Here's how the part is built. I have some questions about the finished solid (model axes, mm). A direction names the side the tool comes from. Coordinates: 2 decimals unless noted, no trailing zeros. Loops run counter-clockwise (first coordinate to the right, second up) from the corner with the lowest first, then second, coordinate; pieces in that order, holes last. Notation, with made-up numbers: (63, 80) -> (107, 80) arc R17 ccw to (107, 108) -> close; hole circle Ø11 at (48.25, 45.5). An arc over 180 degrees is marked (long way). Answer as a JSON object with one key per item and string values. Group by question number.
Q1. On a 3-axis mill with a long thin cutter (end or side, diameter ignored), from which of +Z, -Z, +X, -X, +Y, -Y can I reach the whole of each face in a straight line? I mean faces 4 (the flat face through (24, 0, -5)), 5 (the flat face through (97.93, 6.14, 0.04)), 6 (the flat face through (97.812, -6.107, 0.042)). Say none if no direction works.
Q2. I need wall thicknesses on line 1 (Y direction, x = 104, z = -0.7); line 2 (Y direction, x = 0, z = 3); line 3 (X direction, y = -1, z = 4.25). Which ranges of each line are inside material? Lowest first, please.
Q3. I want a section at D-D on x = 58. Write out the boundary of the cut face in (y, z).
Q4. I'm going to push flat-ended pins straight in: pin 1 (1 mm diameter, centred on y = -15, z = -1.5, fed in from +X); pin 2 (1.6 mm diameter, centred on y = 1.5, z = 3.5, fed in from +X); pin 3 (4.5 mm diameter, centred on x = 96.5, y = 0, fed in from -Z); pin 4 (5.5 mm diameter, centred on x = 104, y = 0, fed in from -Z). Where does each tip first touch, or does it pass through?
Q5. Thinking about a two-plate mould opening in X: for faces 1 (the flat face through (-19.7, 19.9, 0.1)), 2 (the flat face through (64, -5, 0)), 3 (the flat face through (0, 28, 0)), which applies, released by +X, released by -X, zero draft, split by the parting line, or undercut?
Q6. I want a section at A-A on x = 0. Write out the boundary of the cut face in (y, z).
Q7. I want a section at C-C on y = 9.5. Write out the boundary of the cut face in (x, z), then the cut area to 3 significant figures.
Q8. I want a section at B-B on z = -1.25. Write out the boundary of the cut face in (x, y), then the cut area to 3 significant figures.
```python
from build123d import *

# Parameters (mm, degrees)
SKETCH_1_3_R        = 22.5
BOSS_EXTRUDE1_DEPTH = 5
BOSS_EXTRUDE2_DEPTH = 3
SKETCH2_R           = 3
CUT_EXTRUDE1_DEPTH  = 15.5


with BuildPart() as part:
    # Sketch 1_3 → Boss-Extrude1 (new, symmetric)
    with BuildSketch(Plane.XY):
        Polygon((34.597979746, 5), (28, 11.597979746), (11.597979746, 28), (-11.597979746, 28), (-28, 11.597979746), (-28, -11.597979746), (-11.597979746, -28), (11.597979746, -28), (19.798989873, -19.798989873), (28, -11.597979746), (34.597979746, -5), (82, -5), (84, -3), (84, 3), (82, 5), align=None)
        Circle(SKETCH_1_3_R, mode=Mode.SUBTRACT)
    extrude(amount=BOSS_EXTRUDE1_DEPTH, both=True)

    # Sketch 1_3 2 → Boss-Extrude2 (add, symmetric)
    with BuildSketch(Plane.XY):
        with BuildLine():
            Line((93.682479249, 5), (82, 5))
            Line((82, 5), (84, 3))
            Line((84, 3), (84, -3))
            Line((84, -3), (82, -5))
            Line((82, -5), (93.682479249, -5))
            Line((93.682479249, -5), (102.058857162, -7.244443697))
            ThreePointArc((102.058857162, -7.244443697), (111.5, 0), (102.058857162, 7.244443697))
            Line((102.058857162, 7.244443697), (93.682479249, 5))
        make_face()
    extrude(amount=BOSS_EXTRUDE2_DEPTH, both=True)

    # Sketch2 → Cut-Extrude1 (cut, symmetric)
    with BuildSketch(Plane.XY.offset(3)):
        with Locations((104, 0)):
            Circle(SKETCH2_R)
    extrude(amount=CUT_EXTRUDE1_DEPTH, both=True, mode=Mode.SUBTRACT)


solid = part.part
```
Result set:
{
 "1": {"face 4": "-Z, +X, -X, +Y, -Y", "face 5": "+Z, -Z, +Y", "face 6": "+Z, -Z, -Y"},
 "2": {"line 1": "y = -7.5 to -3, 3 to 7.5", "line 2": "y = -28 to -22.5, 22.5 to 28", "line 3": "x = -28 to -22.48, 22.48 to 84"},
 "3": {"outline": "(-5, -5) -> (5, -5) -> (5, 5) -> (-5, 5) -> close"},
 "4": {"pin 1": "stops at x = 25.1", "pin 2": "stops at x = 111.45", "pin 3": "stops at z = -3", "pin 4": "passes through"},
 "5": {"face 1": "released by -X", "face 2": "undercut", "face 3": "zero draft"},
 "6": {"outline": "(-28, -5) -> (-22.5, -5) -> (-22.5, 5) -> (-28, 5) -> close; (22.5, -5) -> (28, -5) -> (28, 5) -> (22.5, 5) -> close"},
 "7": {"outline": "(-28, -5) -> (-20.4, -5) -> (-20.4, 5) -> (-28, 5) -> close; (20.4, -5) -> (30.1, -5) -> (30.1, 5) -> (20.4, 5) -> close", "area": "173 mm²"},
 "8": {"outline": "(-28, -11.6) -> (-11.6, -28) -> (11.6, -28) -> (34.6, -5) -> (93.68, -5) -> (102.06, -7.24) arc R7.5 ccw (long way) to (102.06, 7.24) -> (93.68, 5) -> (34.6, 5) -> (11.6, 28) -> (-11.6, 28) -> (-28, 11.6) -> close; hole circle Ø45 at (0, 0); hole circle Ø6 at (104, 0)", "area": "1,900 mm²"}
}
